from build123d import *

# Parameters (mm, degrees)
BASE_DISC_SKETCH_328_R            = 164
BASE_DISC_328X15_DEPTH            = 15
HUB_SKETCH_164_R                  = 82
HUB_164X54_DEPTH                  = 54
CENTRE_BORE_SKETCH_56_R           = 28
CENTRE_BORE_56_DEPTH              = 242.97727166
CLEVIS_LUG_PROFILE_SKETCH_R       = 7.5
CLEVIS_LUG_DEPTH                  = 22
CLEVIS_SLOT_30_DEPTH              = 30
CLEVIS_LUG_PATTERN_3X_COUNT       = 3
LARGE_HOLE_SKETCH_35_R            = 17.5
LARGE_HOLE_35_DEPTH               = 239.134415824
LARGE_HOLE_PATTERN_3X_35_COUNT    = 3
MOUNTING_HOLE_SKETCH_10_R         = 5
MOUNTING_HOLE_10_DEPTH            = 242.97727166
MOUNTING_HOLE_PATTERN_6X_10_COUNT = 6


with BuildPart() as part:
    # Base Disc Sketch Ø328 → Base Disc Ø328x15 (new body)
    with BuildSketch(Plane(origin=(0, 0, 0), x_dir=(1, 0, 0), z_dir=(0, 1, 0))):
        with Locations(Location((0, 0, 0), (0, 0, 270))):
            Circle(BASE_DISC_SKETCH_328_R)
    extrude(amount=BASE_DISC_328X15_DEPTH)

    # Hub Sketch Ø164 → Hub Ø164x54 (add)
    with BuildSketch(Plane(origin=(0, 15, 0), x_dir=(1, 0, 0), z_dir=(0, 1, 0))):
        with Locations(Location((0, 0, 0), (0, 0, 270))):
            Circle(HUB_SKETCH_164_R)
    extrude(amount=HUB_164X54_DEPTH)

    # Centre Bore Sketch Ø56 → Centre Bore Ø56 (cut, through all)
    with BuildSketch(Plane(origin=(0, 69, 0), x_dir=(1, 0, 0), z_dir=(0, 1, 0))):
        with Locations(Location((0, 0, 0), (0, 0, 270))):
            Circle(CENTRE_BORE_SKETCH_56_R)
    extrude(amount=-CENTRE_BORE_56_DEPTH, mode=Mode.SUBTRACT)

    # Clevis Lug Profile Sketch → Clevis Lug (add, symmetric)
    with BuildSketch(Plane(origin=(0, 0, 0), x_dir=(0, 0, -1), z_dir=(1, 0, 0))):
        with BuildLine():
            Line((-97, 69), (-69.408237338, 69))
            Line((-69.408237338, 69), (-69.408237338, 39))
            Line((-69.408237338, 39), (-97, 39))
            ThreePointArc((-97, 39), (-112, 54), (-97, 69))
        make_face()
        with Locations((-97, 54)):
            Circle(CLEVIS_LUG_PROFILE_SKETCH_R, mode=Mode.SUBTRACT)
    clevis_lug = extrude(amount=CLEVIS_LUG_DEPTH, both=True)

    # Clevis Slot Profile Sketch → Clevis Slot 30 (cut)
    with BuildSketch(Plane(origin=(0, 69, 0), x_dir=(1, 0, 0), z_dir=(0, 1, 0))):
        Polygon((0, -112), (-8, -112), (-8, -78.993670633), (8, -78.993670633), (8, -112), align=None)
    clevis_slot_30 = extrude(amount=-CLEVIS_SLOT_30_DEPTH, mode=Mode.SUBTRACT)

    # Clevis Lug Pattern 3x: Clevis Lug, Clevis Slot 30 ×3 about axis
    clevis_lug_pattern_3x_axis = Axis((0, 0, 0), (0, 1, 0))
    add([clevis_lug.rotate(clevis_lug_pattern_3x_axis, i * 360 / CLEVIS_LUG_PATTERN_3X_COUNT) for i in range(1, CLEVIS_LUG_PATTERN_3X_COUNT)])
    add([clevis_slot_30.rotate(clevis_lug_pattern_3x_axis, i * 360 / CLEVIS_LUG_PATTERN_3X_COUNT) for i in range(1, CLEVIS_LUG_PATTERN_3X_COUNT)], mode=Mode.SUBTRACT)

    # Large Hole Sketch Ø35 → Large Hole Ø35 (cut, through all)
    with BuildSketch(Plane(origin=(0, 15, 0), x_dir=(1, 0, 0), z_dir=(0, 1, 0))):
        with Locations(Location((0, -112, 0), (0, 0, 270))):
            Circle(LARGE_HOLE_SKETCH_35_R)
    large_hole_35 = extrude(amount=-LARGE_HOLE_35_DEPTH, mode=Mode.SUBTRACT)

    # Large Hole Pattern 3xØ35: Large Hole Ø35 ×3 about axis
    large_hole_pattern_3x_35_axis = Axis((0, 0, 0), (0, 1, 0))
    for i in range(1, LARGE_HOLE_PATTERN_3X_35_COUNT):
        add(large_hole_35.rotate(large_hole_pattern_3x_35_axis, i * 360 / LARGE_HOLE_PATTERN_3X_35_COUNT), mode=Mode.SUBTRACT)

    # Mounting Hole Sketch Ø10 → Mounting Hole Ø10 (cut, through all)
    with BuildSketch(Plane(origin=(0, 69, 0), x_dir=(1, 0, 0), z_dir=(0, 1, 0))):
        with Locations(Location((-154, 0, 0), (0, 0, 270))):
            Circle(MOUNTING_HOLE_SKETCH_10_R)
    mounting_hole_10 = extrude(amount=-MOUNTING_HOLE_10_DEPTH, mode=Mode.SUBTRACT)

    # Mounting Hole Pattern 6xØ10: Mounting Hole Ø10 ×6 about axis
    mounting_hole_pattern_6x_10_axis = Axis((0, 0, 0), (0, 1, 0))
    for i in range(1, MOUNTING_HOLE_PATTERN_6X_10_COUNT):
        add(mounting_hole_10.rotate(mounting_hole_pattern_6x_10_axis, i * 360 / MOUNTING_HOLE_PATTERN_6X_10_COUNT), mode=Mode.SUBTRACT)


solid = part.part
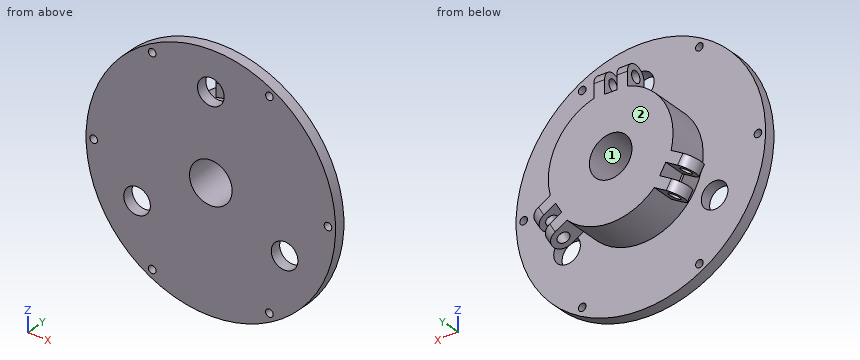
Part model, mm, in its own coordinate system. Face numbers are marked on the shaded views. Round coordinates to 2 decimals unless told otherwise and drop trailing zeros. Write each loop counter-clockwise with the first axis right and the second up, starting at its lowest first coordinate (ties: lowest second). Pieces come first, ordered by that corner, then holes. Notation, with made-up numbers: (37.25, 83.25) - (81.25, 83.25) arc R20 cw to (81.25, 102.25) - close; hole circle Ø1 at (41, 88). An arc over 180 degrees is marked (long way). Use CSV: the item, a comma, the result in double quotes.
Item 1: Slice it at B-B, the plane z = 0. Write the cut outline in (x, y).
Results list:
outline,"(-164, 0) - (-159, 0) - (-159, 15) - (-164, 15) - close; (-149, 0) - (-28, 0) - (-28, 69) - (-82, 69) - (-82, 15) - (-149, 15) - close; (28, 0) - (149, 0) - (149, 15) - (82, 15) - (82, 69) - (28, 69) - close; (159, 0) - (164, 0) - (164, 15) - (159, 15) - close"
Item 2: Wall check: L1, parallel to X at y = 3.75, z = 0; L2, parallel to Y at x = -13.75, z = 97; L3, parallel to X at y = 6, z = -56. Give the ranges that are in metal, low to high.
Results list:
L1,"x = -164 to -159, -149 to -28, 28 to 149, 159 to 164"
L2,"y = 0 to 15, 39 to 46.5, 61.5 to 69"
L3,"x = -154.14 to -114.49, -79.49 to 79.49, 114.49 to 154.14"
Item 3: Flat gauge pins, fed straight in: P1, Ø4, axis at x = 38.5, y = 34.5, coming from the +Z side; P2, Ø2, axis at y = 59.5, z = -16, coming from the +X side; P3, Ø5, axis at y = 53, z = 22.5, coming from the +X side; P4, Ø1, axis at y = 42, z = -83, coming from the +X side. Where does each tip first touch, or does it go through?
Results list:
P1,"stops at z = 73.43"
P2,"stops at x = 80.62"
P3,"stops at x = 79.52"
P4,"passes through"
Item 4: Pull direction X, two halves, no side cores. Call the marked faces 1 and 2: pulls with the +X half, pulls with the -X half, needs draft (parallel to the pull), parting line crosses it, or undercut.
Results list:
face 1,"undercut"
face 2,"needs draft"
Item 5: Slice it at D-D, the plane z = 51. Write the cut outline in (x, y).
Results list:
outline,"(-155.87, 0) - (155.87, 0) - (155.87, 15) - (64.21, 15) - (64.21, 69) - (-64.21, 69) - (-64.21, 15) - (-155.87, 15) - close"
Item 6: Slice it at C-C, the plane y = 24. Write the cut outline in (x, z).
Results list:
outline,"circle Ø164 at (0, 0); hole circle Ø56 at (0, 0)"
Item 7: Slice it at A-A, the plane x = 0. Write the cut outline in (y, z).
Results list:
outline,"(0, -164) - (15, -164) - (15, -82) - (69, -82) - (69, -28) - (0, -28) - close; (0, 28) - (69, 28) - (69, 78.99) - (39, 78.99) - (39, 82) - (15, 82) - (15, 94.5) - (0, 94.5) - close; (0, 129.5) - (15, 129.5) - (15, 164) - (0, 164) - close"
